Input: part model. Units: mm. Frame: model coordinates. Face numbers are marked on the shaded views. A direction names the side the tool comes from. Round coordinates to 2 decimals unless told otherwise and drop trailing zeros. Loops run counter-clockwise (first coordinate to the right, second up) from the corner with the lowest first, then second, coordinate; pieces in that order, holes last. Notation, with made-up numbers: (73, 3.5) - (77, 3.5) arc R19 cw to (77, 22.5) - close; hole circle Ø3 at (47.25, 65). An arc over 180 degrees is marked (long way). Use CSV: the item, a comma, the result in double quotes. Start each with the question number.
1. Cut plane D-D (y = 20). Return loops of the section in (x, z), and give its area (3 significant figures).
2. Cut plane B-B (y = -25). Return loops of the section in (x, z), and give its area (3 significant figures).
3. Cut plane A-A (z = 14). Give the number of separate pieces and of enclosed holes in the cut face, and give its area (3 significant figures).
4. Cut plane C-C (x = -3). Return loops of the section in (y, z).
5. Material intervals for probe 1 along X at (y, z) = (-27.9, 5.5); probe 2 along X at (y, z) = (-22, 20.25); probe 3 along X at (y, z) = (-16, 21.5), sorted ascending. Write a range as from..to.
6. Pin query (flat end, axial travel): P1, Ø1.9, axis at x = 25.5, z = 24.5, coming from the +Y side; P2, Ø10.5, axis at y = 21.5, z = 19, coming from the +X side; P3, Ø4.5, axis at y = 22.74, z = 6, coming from the +X side. Return the tip coordinate at first contact, or that it passes through.
7. Access query for the marked faces 1, 2 and 3. Directions: +Z, -Z, +X, -X, +Y, -Y. A direction counts if a zero-diameter tool reaches every point of the face in a straight line with its end or side. Return the directions, or none.
```python
from build123d import *

# Parameters (mm, degrees)
CLAMP_BODY_DEPTH             = 28
SIDE_RECESS_A_DEPTH          = 18
SIDE_RECESS_B_DEPTH          = 18
LOWER_START                  = -28
LOWER_SIDE_BOSS_DEPTH        = 28
LOWER_BOSS_RELIEF_A_DEPTH    = 11
LOWER_START_2                = -11
LOWER_BOSS_RELIEF_B_DEPTH    = 11
UPPER_SIDE_BOSS_DEPTH        = 28
UPPER_BOSS_RELIEF_A_DEPTH    = 11
UPPER_START                  = -11
UPPER_BOSS_RELIEF_B_DEPTH    = 11
CLAMP_SCREW_HOLES_SKETCH_R   = 2
CLAMP_SCREW_HOLES_3X_DEPTH   = 20
FOOT_MOUNTING_HOLES_SKETCH_R = 2
FOOT_MOUNTING_HOLES_DEPTH    = 20


with BuildPart() as part:
    # Clamp Body Profile → Clamp Body (new body)
    with BuildSketch(Plane.XY):
        with BuildLine():
            Line((-20, 0), (-20, -22.4))
            ThreePointArc((-20, -22.4), (-20.46862915, -23.53137085), (-21.6, -24))
            Line((-21.6, -24), (-28, -24))
            Line((-28, -24), (-28, -30))
            Line((-28, -30), (-15.6, -30))
            Line((-15.6, -30), (-15.6, -28.4))
            Line((-15.6, -28.4), (-14, -28.4))
            Line((-14, -28.4), (-14, -14.282856857))
            ThreePointArc((-14, -14.282856857), (0, -20), (14, -14.282856857))
            Line((14, -14.282856857), (14, -28.4))
            Line((14, -28.4), (15.6, -28.4))
            Line((15.6, -28.4), (15.6, -30))
            Line((15.6, -30), (28, -30))
            Line((28, -30), (28, -24))
            Line((28, -24), (21.6, -24))
            ThreePointArc((21.6, -24), (20.46862915, -23.53137085), (20, -22.4))
            Line((20, -22.4), (20, 0))
            ThreePointArc((20, 0), (16.431676725, 11.401754251), (7, 18.734993995))
            Line((7, 18.734993995), (7, 27.174984355))
            Line((7, 27.174984355), (1, 27.174984355))
            Line((1, 27.174984355), (1, 19.974984355))
            Line((1, 19.974984355), (1, 13.964240044))
            ThreePointArc((1, 13.964240044), (0, -14), (-1, 13.964240044))
            Line((-1, 13.964240044), (-1, 19.974984355))
            Line((-1, 19.974984355), (-1, 27.174984355))
            Line((-1, 27.174984355), (-7, 27.174984355))
            Line((-7, 27.174984355), (-7, 18.734993995))
            ThreePointArc((-7, 18.734993995), (-16.431676725, 11.401754251), (-20, 0))
        make_face()
    extrude(amount=CLAMP_BODY_DEPTH)

    # Side Recess A Sketch → Side Recess A (cut)
    with BuildSketch(Plane(origin=(7, 0, 0), x_dir=(0, 0, -1), z_dir=(1, 0, 0))):
        with BuildLine():
            Line((-28, 26.374984355), (-28, 27.174984355))
            Line((-28, 27.174984355), (-27.2, 27.174984355))
            ThreePointArc((-27.2, 27.174984355), (-27.765685425, 26.94066978), (-28, 26.374984355))
        make_face()
    extrude(amount=-SIDE_RECESS_A_DEPTH, mode=Mode.SUBTRACT)

    # Side Recess B Sketch → Side Recess B (cut)
    with BuildSketch(Plane(origin=(7, 0, 0), x_dir=(0, 0, -1), z_dir=(1, 0, 0))):
        with BuildLine():
            Line((0, 27.174984355), (0, 26.374984355))
            ThreePointArc((0, 26.374984355), (-0.234314575, 26.94066978), (-0.8, 27.174984355))
            Line((-0.8, 27.174984355), (0, 27.174984355))
        make_face()
    extrude(amount=-SIDE_RECESS_B_DEPTH, mode=Mode.SUBTRACT)

    # Lower Side Boss Sketch → Lower Side Boss (add)
    with BuildSketch(Plane.XY.offset(28).offset(LOWER_START)):
        with BuildLine():
            Line((20, 0), (28, -24))
            Line((28, -24), (21.6, -24))
            ThreePointArc((21.6, -24), (20.46862915, -23.53137085), (20, -22.4))
            Line((20, -22.4), (20, 0))
        make_face()
    extrude(amount=LOWER_SIDE_BOSS_DEPTH)

    # Lower Boss Relief A Sketch → Lower Boss Relief A (cut)
    with BuildSketch(Plane.XY.offset(28)):
        with BuildLine():
            Line((20, 0), (28, -24))
            Line((28, -24), (21.6, -24))
            ThreePointArc((21.6, -24), (20.46862915, -23.53137085), (20, -22.4))
            Line((20, -22.4), (20, 0))
        make_face()
    extrude(amount=-LOWER_BOSS_RELIEF_A_DEPTH, mode=Mode.SUBTRACT)

    # Lower Boss Relief B Sketch → Lower Boss Relief B (cut)
    with BuildSketch(Plane(origin=(0, 0, 0), x_dir=(-1, 0, 0), z_dir=(0, 0, -1)).offset(LOWER_START_2)):
        with BuildLine():
            Line((-20, 0), (-20, -22.4))
            ThreePointArc((-20, -22.4), (-20.46862915, -23.53137085), (-21.6, -24))
            Line((-21.6, -24), (-28, -24))
            Line((-28, -24), (-20, 0))
        make_face()
    extrude(amount=LOWER_BOSS_RELIEF_B_DEPTH, mode=Mode.SUBTRACT)

    # Upper Side Boss Sketch → Upper Side Boss (add)
    with BuildSketch(Plane(origin=(0, 0, 0), x_dir=(-1, 0, 0), z_dir=(0, 0, -1))):
        with BuildLine():
            Line((20, 0), (28, -24))
            Line((28, -24), (21.6, -24))
            ThreePointArc((21.6, -24), (20.46862915, -23.53137085), (20, -22.4))
            Line((20, -22.4), (20, 0))
        make_face()
    extrude(amount=-UPPER_SIDE_BOSS_DEPTH)

    # Upper Boss Relief A Sketch → Upper Boss Relief A (cut)
    with BuildSketch(Plane(origin=(0, 0, 0), x_dir=(-1, 0, 0), z_dir=(0, 0, -1))):
        with BuildLine():
            Line((20, 0), (20, -22.4))
            ThreePointArc((20, -22.4), (20.46862915, -23.53137085), (21.6, -24))
            Line((21.6, -24), (28, -24))
            Line((28, -24), (20, 0))
        make_face()
    extrude(amount=-UPPER_BOSS_RELIEF_A_DEPTH, mode=Mode.SUBTRACT)

    # Upper Boss Relief B Sketch → Upper Boss Relief B (cut)
    with BuildSketch(Plane.XY.offset(28).offset(UPPER_START)):
        with BuildLine():
            Line((-20, 0), (-20, -22.4))
            ThreePointArc((-20, -22.4), (-20.46862915, -23.53137085), (-21.6, -24))
            Line((-21.6, -24), (-28, -24))
            Line((-28, -24), (-20, 0))
        make_face()
    extrude(amount=UPPER_BOSS_RELIEF_B_DEPTH, mode=Mode.SUBTRACT)

    # Clamp Screw Holes Sketch → Clamp Screw Holes 3x (cut)
    with BuildSketch(Plane(origin=(7, 0, 0), x_dir=(0, 0, -1), z_dir=(1, 0, 0))):
        with Locations((-22, 22.743733378)):
            Circle(CLAMP_SCREW_HOLES_SKETCH_R)
        with Locations((-14, 22.743733378)):
            Circle(CLAMP_SCREW_HOLES_SKETCH_R)
        with Locations((-6, 22.743733378)):
            Circle(CLAMP_SCREW_HOLES_SKETCH_R)
    extrude(amount=-CLAMP_SCREW_HOLES_3X_DEPTH, mode=Mode.SUBTRACT)

    # Foot Mounting Holes Sketch → Foot Mounting Holes (cut)
    with BuildSketch(Plane(origin=(0, -24, 0), x_dir=(1, 0, 0), z_dir=(0, 1, 0))):
        with Locations(Location((24.8, -22.5, 0), (0, 0, 270))):
            Circle(FOOT_MOUNTING_HOLES_SKETCH_R)
        with Locations(Location((24.8, -5.5, 0), (0, 0, 270))):
            Circle(FOOT_MOUNTING_HOLES_SKETCH_R)
        with Locations(Location((-24.8, -5.5, 0), (0, 0, 270))):
            Circle(FOOT_MOUNTING_HOLES_SKETCH_R)
        with Locations(Location((-24.8, -22.5, 0), (0, 0, 270))):
            Circle(FOOT_MOUNTING_HOLES_SKETCH_R)
    extrude(amount=-FOOT_MOUNTING_HOLES_DEPTH, mode=Mode.SUBTRACT)


solid = part.part
```
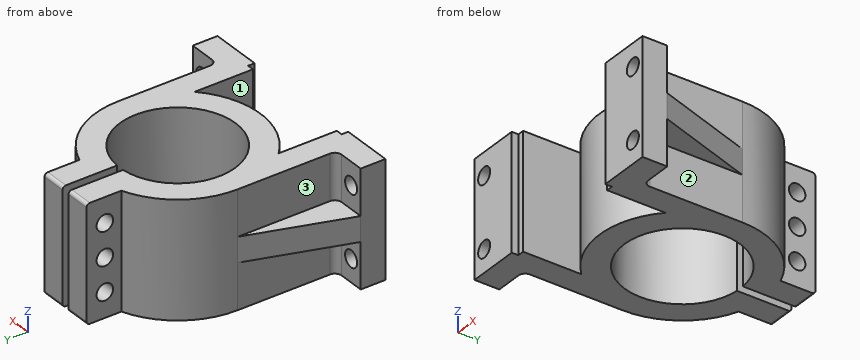
Established:
1,outline,"(-7, 0) - (-1, 0) - (-1, 28) - (-7, 28) - close; (1, 0) - (7, 0) - (7, 28) - (1, 28) - close"
1,area,"336 mm2"
2,outline,"(-28, 0) - (-14, 0) - (-14, 28) - (-28, 28) - close; (14, 0) - (28, 0) - (28, 28) - (14, 28) - close; hole circle Ø4 at (-24.8, 5.5); hole circle Ø4 at (-24.8, 22.5); hole circle Ø4 at (24.8, 5.5); hole circle Ø4 at (24.8, 22.5)"
2,area,"734 mm2"
3,separate pieces,"3"
3,enclosed holes,"0"
3,area,"1,200 mm2"
4,outline,"(-19.77, 0) - (-13.67, 0) - (-13.67, 28) - (-19.77, 28) - close; (13.67, 0) - (26.37, 0) arc R0.8 ccw to (27.17, 0.8) - (27.17, 27.2) arc R0.8 ccw to (26.37, 28) - (13.67, 28) - close; hole circle Ø4 at (22.74, 6); hole circle Ø4 at (22.74, 14); hole circle Ø4 at (22.74, 22)"
5,probe 1,"x = -28..-26.8, -22.8..-14, 14..22.8, 26.8..28"
5,probe 2,"x = -20..-14, 14..20"
5,probe 3,"x = -20..-14, -12..12, 14..20"
6,P1,"stops at y = -24"
6,P2,"stops at x = 11.66"
6,P3,"stops at x = 7"
7,face 1,"+Z, -Z, -Y"
7,face 2,"-Z, +X, +Y"
7,face 3,"+Z, -X, +Y"
